Source: CAD feature listing. Evaluate the final solid. Frame: model axes, mm. Face numbers are marked on the shaded views. A direction names the side the tool comes from. Give positions to 0.01 mm unless a question says otherwise; leave off trailing zeros. Order: outer loops, then holes, each group sorted by start corner. A loop starts at its lowest first (then second) coordinate and runs counter-clockwise, first axis right, second up. Notation, with made-up numbers: M 64.5,19.5 L 73.5,19.5 A26 cw 73.5,49.5 Z; hole C -10.5,84 d1. An arc over 180 degrees is marked long. Return JSON: item names as keys, results as strings.
from build123d import *

# Parameters (mm, degrees)
SKETCH1_W                                            = 116
SKETCH1_H                                            = 30
BOSS_EXTRUDE1_DEPTH                                  = 10
CUT_EXTRUDE2_DEPTH                                   = 64.158530699
HOLE_SIZE_PER_SOCKET_HEAD_CAP_SCREW_TYPE_D           = 4.5
HOLE_SIZE_PER_SOCKET_HEAD_CAP_SCREW_TYPE_DEPTH       = 14.5
HOLE_SIZE_PER_SOCKET_HEAD_CAP_SCREW_TYPE_CBORE_D     = 8
HOLE_SIZE_PER_SOCKET_HEAD_CAP_SCREW_TYPE_CBORE_DEPTH = 4.6
M4_TAPPED_HOLE1_D                                    = 3.3
F_5_0_5_DIAMETER_HOLE1_D                             = 5
F_5_0_5_DIAMETER_HOLE1_DEPTH                         = 7
F_5_0_5_DIAMETER_HOLE1_TIP                           = 1.502151548
M4_TAPPED_HOLE2_AT_2_COUNT                           = 2
M4_TAPPED_HOLE2_AT_2_PITCH                           = 80
CHAMFER1_SIZE                                        = 4
M4_TAPPED_HOLE3_D                                    = 3.3
M4_TAPPED_HOLE3_DEPTH                                = 10.1
M4_TAPPED_HOLE3_TIP                                  = 0.991420021
CUT_EXTRUDE3_DEPTH                                   = 67.060578275
SKETCH18_W                                           = 20
SKETCH18_H                                           = 20
CUT_EXTRUDE4_DEPTH                                   = 64.158530699
SKETCH19_W                                           = 28
SKETCH19_H                                           = 24
CUT_EXTRUDE5_DEPTH                                   = 1.5
FILLET1_R                                            = 3
M3_TAPPED_HOLE1_D                                    = 2.5
M3_TAPPED_HOLE1_DEPTH                                = 7.5
M3_TAPPED_HOLE1_TIP                                  = 0.751075774
CHAMFER2_SIZE                                        = 1
CHAMFER2_SIZE2                                       = 1.04665043
CHAMFER3_SIZE                                        = 1


with BuildPart() as part:
    # Sketch1 → Boss-Extrude1 (new, symmetric)
    with BuildSketch(Plane(origin=(0, 0, 0), x_dir=(1, 0, 0), z_dir=(0, 1, 0))):
        Rectangle(SKETCH1_W, SKETCH1_H)
    extrude(amount=BOSS_EXTRUDE1_DEPTH, both=True)

    # Sketch3 → Cut-Revolve1 (revolve, cut)
    with BuildSketch(Plane.XY):
        Polygon((-39.473720558, -128.867912183), (58.526279442, 40.873066959), (49, 46.373066959), (-49, -123.367912183), align=None)
    revolve(axis=Axis((28, 10, 0), (-0.5000000000000041, -0.8660254037844363, 0)), mode=Mode.SUBTRACT)

    # Sketch4 → Cut-Extrude2 (cut, through all)
    with BuildSketch(Plane(origin=(0, 10, 0), x_dir=(1, 0, 0), z_dir=(0, 1, 0))):
        with BuildLine():
            Line((6, 0.5), (58, 0.5))
            Line((58, 0.5), (58, -0.5))
            Line((58, -0.5), (6, -0.5))
            ThreePointArc((6, -0.5), (5.5, 0), (6, 0.5))
        make_face()
    extrude(amount=-CUT_EXTRUDE2_DEPTH, mode=Mode.SUBTRACT)

    # Hole size per socket head cap screw type1
    with Locations(Plane.XY.offset(15)):
        with Locations((53, 4)):
            CounterBoreHole(HOLE_SIZE_PER_SOCKET_HEAD_CAP_SCREW_TYPE_D / 2, HOLE_SIZE_PER_SOCKET_HEAD_CAP_SCREW_TYPE_CBORE_D / 2, HOLE_SIZE_PER_SOCKET_HEAD_CAP_SCREW_TYPE_CBORE_DEPTH, depth=HOLE_SIZE_PER_SOCKET_HEAD_CAP_SCREW_TYPE_DEPTH)

    # M4 Tapped Hole1 (through all)
    with Locations(Plane.XY.offset(-0.5)):
        with Locations((53, 4)):
            Hole(M4_TAPPED_HOLE1_D / 2)

    # Ø5.0 (5) Diameter Hole1
    with Locations(Plane(origin=(0, 0, -15), x_dir=(-1, 0, 0), z_dir=(0, 0, -1))):
        with Locations((-53, 4)):
            Hole(F_5_0_5_DIAMETER_HOLE1_D / 2, depth=F_5_0_5_DIAMETER_HOLE1_DEPTH)
            with Locations((0, 0, -(F_5_0_5_DIAMETER_HOLE1_DEPTH + F_5_0_5_DIAMETER_HOLE1_TIP / 2))):  # 118° drill point
                Cone(0, F_5_0_5_DIAMETER_HOLE1_D / 2, F_5_0_5_DIAMETER_HOLE1_TIP, mode=Mode.SUBTRACT)

    # Sketch11 → M4 Tapped Hole2 (revolve, cut)
    with BuildSketch(Plane(origin=(-38, 5.5, 15), x_dir=(0, -1, 0), z_dir=(1, 0, 0))):
        Polygon((0, 0), (0, 11.091420021), (1.65, 10.1), (1.65, 0), align=None)
    m4_tapped_hole2 = revolve(axis=Axis((-38, 5.5, 21.35), (0, 0, -1)), mode=Mode.SUBTRACT)

    # M4 Tapped Hole2 at 2: M4 Tapped Hole2 ×2
    with Locations(*[(i * M4_TAPPED_HOLE2_AT_2_PITCH, 0, 0) for i in range(1, M4_TAPPED_HOLE2_AT_2_COUNT)]):
        add(m4_tapped_hole2, mode=Mode.SUBTRACT)

    # Mirror1: M4 Tapped Hole2 across plane
    add(m4_tapped_hole2.mirror(Plane.XY), mode=Mode.SUBTRACT)

    # Mirror1 copy 1 sketch → Mirror1 copy 1 (revolve, cut)
    with BuildSketch(Plane(origin=(42, 5.5, -15), x_dir=(0, -1, 0), z_dir=(1, 0, 0))):
        Polygon((0, 0), (0, -11.091420021), (1.65, -10.1), (1.65, 0), align=None)
    revolve(axis=Axis((42, 5.5, -21.35), (0, 0, -1)), mode=Mode.SUBTRACT)

    # Chamfer1
    chamfer1_edges = [part.edges().sort_by_distance(p)[0] for p in [
        (-58, 10, 0),
    ]]
    chamfer(chamfer1_edges, length=CHAMFER1_SIZE)

    # M4 Tapped Hole3
    with Locations(Plane(origin=(58, 0, 0), x_dir=(0, 0, -1), z_dir=(1, 0, 0))):
        with Locations((-12, -3), (12, -3)):
            Hole(M4_TAPPED_HOLE3_D / 2, depth=M4_TAPPED_HOLE3_DEPTH)
            with Locations((0, 0, -(M4_TAPPED_HOLE3_DEPTH + M4_TAPPED_HOLE3_TIP / 2))):  # 118° drill point
                Cone(0, M4_TAPPED_HOLE3_D / 2, M4_TAPPED_HOLE3_TIP, mode=Mode.SUBTRACT)

    # Sketch17 → Cut-Extrude3 (cut, through all)
    with BuildSketch(Plane.XY.offset(15)):
        Polygon((-58, -10), (56, -10), (56, -6.977347492), (-58, -2), align=None)
    extrude(amount=-CUT_EXTRUDE3_DEPTH, mode=Mode.SUBTRACT)

    # Sketch18 → Cut-Extrude4 (cut, through all)
    with BuildSketch(Plane(origin=(0, 10, 0), x_dir=(1, 0, 0), z_dir=(0, 1, 0))):
        with Locations((-38, 0)):
            Rectangle(SKETCH18_W, SKETCH18_H)
    extrude(amount=-CUT_EXTRUDE4_DEPTH, mode=Mode.SUBTRACT)

    # Sketch19 → Cut-Extrude5 (cut)
    with BuildSketch(Plane(origin=(0, 10, 0), x_dir=(1, 0, 0), z_dir=(0, 1, 0))):
        with Locations((-35.5, 0)):
            Rectangle(SKETCH19_W, SKETCH19_H)
    extrude(amount=-CUT_EXTRUDE5_DEPTH, mode=Mode.SUBTRACT)

    # Fillet1
    fillet1_edges = [part.edges().sort_by_distance(p)[0] for p in [
        (-48, 3.031695285, 10),
        (-48, 3.031695285, -10),
        (-28, 2.595085856, -10),
        (-28, 2.595085856, 10),
        (-49.5, 9.25, 12),
        (-49.5, 9.25, -12),
        (-21.5, 9.25, -12),
        (-21.5, 9.25, 12),
    ]]
    fillet(fillet1_edges, radius=FILLET1_R)

    # M3 Tapped Hole1
    with Locations(Plane(origin=(0, 8.5, 0), x_dir=(1, 0, 0), z_dir=(0, 1, 0))):
        with Locations((-25, 6), (-25, -6)):
            Hole(M3_TAPPED_HOLE1_D / 2, depth=M3_TAPPED_HOLE1_DEPTH)
            with Locations((0, 0, -(M3_TAPPED_HOLE1_DEPTH + M3_TAPPED_HOLE1_TIP / 2))):  # 118° drill point
                Cone(0, M3_TAPPED_HOLE1_D / 2, M3_TAPPED_HOLE1_TIP, mode=Mode.SUBTRACT)

    # Chamfer2
    chamfer2_edges = [part.edges().sort_by_distance(p)[0] for p in [
        (-58, -2, 0),
    ]]
    chamfer2_side = [part.faces().sort_by_distance(p)[0] for p in [
        (0.861914044, -4.569966669, 0),
    ]]
    chamfer(chamfer2_edges, length=CHAMFER2_SIZE, length2=CHAMFER2_SIZE2, reference=chamfer2_side[0])

    # Chamfer3
    chamfer3_edges = [part.edges().sort_by_distance(p)[0] for p in [
        (42, 7.15, 15),
        (-38, 7.15, 15),
        (42, 7.15, -15),
        (-38, 7.15, -15),
    ]]
    chamfer(chamfer3_edges, length=CHAMFER3_SIZE)


solid = part.part
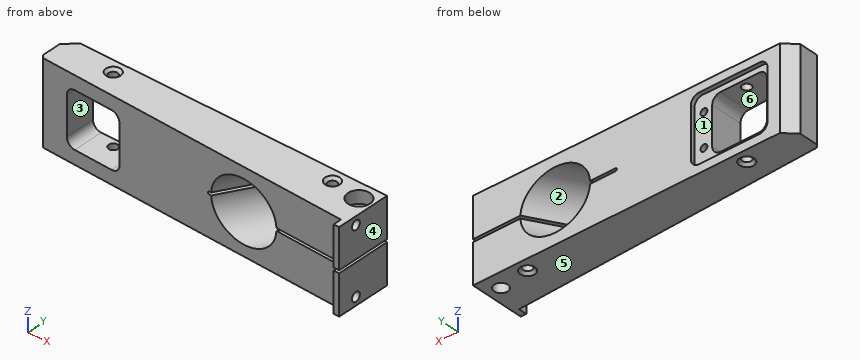
1. Section query A-A (z = 2). Return loops of the section in (x, y), then the cut area to 3 significant figures.
Evaluation:
{"outline": "M -58,-0.95 L -57,-2.04 L -48,-2.44 L -48,8.5 L -49.5,8.5 L -49.5,10 L -54,10 L -58,6 Z; M -28,-3.31 L 6.94,-4.84 L 15.51,10 L -21.5,10 L -21.5,8.5 L -28,8.5 Z; M 31.31,-5.9 L 56,-6.98 L 56,-10 L 58,-10 L 58,10 L 40.49,10 Z; hole C 53,4 d4.5", "area": "1,010 mm^2"}
2. Section query B-B (x = -7). Return loops of the section in (y, z).
Evaluation:
{"outline": "M -4.23,-15 L 10,-15 L 10,15 L -4.23,15 Z"}
3. Ray query, probe 1 along Y at (x, z) = (50, 12); probe 2 along X at (y, z) = (5, -4); probe 3 along X at (y, z) = (-0.5, -7). Return the intervals inside material, ascending.
Evaluation:
{"probe 1": "y = -6.72 to -4.65, -1.35 to 1.35, 6.65 to 10", "probe 2": "x = -58 to -48, -28 to 13.28, 36.95 to 51.69, 54.31 to 58", "probe 3": "x = -58 to -48, -28 to 12.14, 31.74 to 58"}
4. Draft query along X for the marked faces 4, 5 and 6. Return one class per face: pulls with the +X half, pulls with the -X half, needs draft (parallel to the pull), parting line crosses it, or undercut.
Evaluation:
{"face 4": "pulls with the +X half", "face 5": "needs draft", "face 6": "undercut"}
5. Set-up query: the marked faces 1, 2 and 3. Return all of +Z, -Z, +X, -X, +Y, -Y with unobstructed straight access to the full face (end or side cutting, diameter ignored); none if empty.
Evaluation:
{"face 1": "+Y", "face 2": "none", "face 3": "+Y, -Y"}
6. First-contact query: pin 1 (4.5 mm diameter, centred on x = 53, y = 4, fed in from -Z); pin 2 (2 mm diameter, centred on x = -25, z = 6, fed in from +Y); pin 3 (0.9 mm diameter, centred on y = -8.5, z = 7.5, fed in from -X). Flat tips, straight axial feed; report the tip coordinate or a pass-through.
Evaluation:
{"pin 1": "stops at z = -7.85", "pin 2": "stops at y = 0.85", "pin 3": "stops at x = 56"}
